Part model, mm, in its own coordinate system. A direction names the side the tool comes from. Round coordinates to 2 decimals unless told otherwise and drop trailing zeros. Order: outer loops, then holes, each group sorted by start corner. A loop starts at its lowest first (then second) coordinate and runs counter-clockwise, first axis right, second up. Notation, with made-up numbers: (14.25, 51.25) - (49.25, 51.25) arc R29 ccw to (49.25, 83.25) - close; hole circle Ø2 at (32.25, -4). An arc over 180 degrees is marked (long way). Return JSON: item names as keys, results as strings. Group by question number.
Item 1: Probe probe 1 along X at (y, z) = (200, -2); probe 2 along Y at (x, z) = (70, -2.2); probe 3 along Y at (x, z) = (-70, -0.55). List the from-to ranges inside material, lowest first.
Item 2: Two-plate mould, pull along Y, no slides. Class faces 4 (the face through (3.21, -127.703, -149.421)), 5 (the face through (200.455, 2.476, -113.421)), 6 (the face through (-3, -200, -3)): released by +Y, released by -Y, zero draft, split by the parting line, or undercut.
Item 3: Saw through at D-D on z = -160.5. List the corners of the cut face in (x, y) (3 decimals), and give its area (3 significant figures).
Item 4: Saw through at B-B on x = -24.5. List the corners of the cut face in (y, z), and give its area (3 significant figures).
Item 5: Tool access for faces 1 (the face through (-1, 180, 0)), 2 (the face through (-3, 200, -3)), 3 (the face through (-200.455, -2.476, -113.421)): list every direction of +Z, -Z, +X, -X, +Y, -Y with a clear straight run to the whole face (end or side of a thin tool).
Item 6: Saw through at A-A on y = 16.5. List the corners of the cut face in (x, z), and give its area (3 significant figures).
Item 7: Saw through at C-C on z = -221.5. List the corners of the cut face in (x, y) (3 decimals), and give its area (3 significant figures).
Item 8: Drop flat-ended pins along their axis: pin 1 (2.5 mm diameter, centred on y = 5, z = -298.5, fed in from -X); pin 2 (1 mm diameter, centred on y = 22.5, z = -248, fed in from +X); pin 3 (0.9 mm diameter, centred on x = 1.5, z = -299, fed in from -Y); pin 4 (9 mm diameter, centred on x = -210, y = -200, fed in from +Z). Give the stop position or say it passes through.
```python
from build123d import *

# Parameters (mm, degrees)
SKETCH1_W                = 460
SKETCH1_H                = 360
BOSS_EXTRUDE1_DEPTH      = 300
CUT_EXTRUDE1_DEPTH       = 578.927331072
CUT_EXTRUDE3_DEPTH       = 302
SHELL1_T                 = -3
SKETCH7_W                = 315.23883128
SKETCH7_H                = 145.74311397
CUT_EXTRUDE4_DEPTH       = 417.544115311
SKETCH8_W                = 460
SKETCH8_H                = 40
BOSS_EXTRUDE2_DEPTH      = 3
BOSS_EXTRUDE3_REACH      = 524.015
SKETCH9_W                = 460
SKETCH9_H                = 3
SKETCH10_W               = 460
SKETCH10_H               = 40
BOSS_EXTRUDE4_DEPTH      = 3
BOSS_EXTRUDE5_REACH      = 552.364
SKETCH11_W               = 460
SKETCH11_H               = 3
F_7_0_7_DIAMETER_HOLE1_D = 7
LPATTERN1_COUNT          = 4
LPATTERN1_PITCH          = 140
MIRROR5_COPY_1_D         = 7
MIRROR5_COPY_2_D         = 7
MIRROR5_COPY_3_D         = 7


with BuildPart() as part:
    # Sketch1 → Boss-Extrude1 (new body)
    with BuildSketch(Plane.XY):
        Rectangle(SKETCH1_W, SKETCH1_H)
    extrude(amount=-BOSS_EXTRUDE1_DEPTH)

    # Sketch3 → Cut-Extrude1 (cut, through all)
    with BuildSketch(Plane(origin=(230, 0, 0), x_dir=(0, 0, -1), z_dir=(1, 0, 0))):
        Polygon((0, 180), (300, 75), (300, 180), align=None)
        Polygon((300, -180), (0, -180), (300, -75), align=None)
    extrude(amount=-CUT_EXTRUDE1_DEPTH, mode=Mode.SUBTRACT)

    # Sketch6 → Cut-Extrude3 (cut, symmetric)
    with BuildSketch(Plane(origin=(0, 0, 0), x_dir=(1, 0, 0), z_dir=(0, 1, 0))):
        Polygon((-230, 0), (-160, 300), (-230, 300), align=None)
        Polygon((230, 300), (230, 0), (160, 300), align=None)
    extrude(amount=CUT_EXTRUDE3_DEPTH, both=True, mode=Mode.SUBTRACT)

    # Shell1
    shell1_openings = [part.faces().sort_by_distance(p)[0] for p in [
        (0, 0, 0),
    ]]
    offset(amount=SHELL1_T, openings=shell1_openings, kind=Kind.INTERSECTION)

    # Sketch7 → Cut-Extrude4 (cut, through all)
    with BuildSketch(Plane.XY.offset(-297)):
        Rectangle(SKETCH7_W, SKETCH7_H)
    extrude(amount=-CUT_EXTRUDE4_DEPTH, mode=Mode.SUBTRACT)

    # Boss-Extrude3: up to this face of the body (flat: up to its plane)
    boss_extrude3_end = Plane(part.part.faces().sort_by_distance((0, -130.641025641, -141.025641026))[0])
    # Sketch9 → Boss-Extrude3 (add, up to the picked face)
    with BuildSketch(Plane(origin=(0, -180, 0), x_dir=(1, 0, 0), z_dir=(0, 1, 0)), mode=Mode.PRIVATE) as boss_extrude3_sk1:
        with Locations((0, 1.5)):
            Rectangle(SKETCH9_W, SKETCH9_H)
    boss_extrude3_tool1 = split(extrude(boss_extrude3_sk1.sketch, amount=BOSS_EXTRUDE3_REACH, mode=Mode.PRIVATE), bisect_by=boss_extrude3_end, keep=Keep.BOTH, mode=Mode.PRIVATE)


with BuildPart() as body_2:
    # Sketch8 → Boss-Extrude2 (new body)
    with BuildSketch(Plane.XY):
        with Locations((0, -200)):
            Rectangle(SKETCH8_W, SKETCH8_H)
    extrude(amount=-BOSS_EXTRUDE2_DEPTH)


with BuildPart() as part_1:
    add(part.part)

    add(body_2.part)  # Boss-Extrude3 merges body 2
    add(boss_extrude3_tool1.solids().sort_by(Axis((0, -180, -1.5), (0, 1, 0)))[0])

    # Boss-Extrude5: up to this face of the body (flat: up to its plane)
    boss_extrude5_end = Plane(part_1.part.faces().sort_by_distance((0, 130.641025641, -141.025641026))[0])
    # Sketch11 → Boss-Extrude5 (add, up to the picked face)
    with BuildSketch(Plane.XZ.offset(-180), mode=Mode.PRIVATE) as boss_extrude5_sk1:
        with Locations((0, -1.5)):
            Rectangle(SKETCH11_W, SKETCH11_H)
    boss_extrude5_tool1 = split(extrude(boss_extrude5_sk1.sketch, amount=BOSS_EXTRUDE5_REACH, mode=Mode.PRIVATE), bisect_by=boss_extrude5_end, keep=Keep.BOTH, mode=Mode.PRIVATE)


with BuildPart() as body_2_2:
    # Sketch10 → Boss-Extrude4 (new body)
    with BuildSketch(Plane.XY):
        with Locations((0, 200)):
            Rectangle(SKETCH10_W, SKETCH10_H)
    extrude(amount=-BOSS_EXTRUDE4_DEPTH)


with BuildPart() as part_2:
    add(part_1.part)

    add(body_2_2.part)  # Boss-Extrude5 merges body 2 2
    add(boss_extrude5_tool1.solids().sort_by(Axis((0, 180, -1.5), (0, -1, 0)))[0])

    # Ø7.0 (7) Diameter Hole1 (through all)
    with Locations(Plane.XY):
        with Locations((-210, 200)):
            f_7_0_7_diameter_hole1 = Hole(F_7_0_7_DIAMETER_HOLE1_D / 2)

    # LPattern1: Ø7.0 (7) Diameter Hole1 ×4
    with Locations(*[(i * LPATTERN1_PITCH, 0, 0) for i in range(1, LPATTERN1_COUNT)]):
        add(f_7_0_7_diameter_hole1, mode=Mode.SUBTRACT)

    # Mirror5: Ø7.0 (7) Diameter Hole1 across plane
    add(f_7_0_7_diameter_hole1.mirror(Plane.ZX), mode=Mode.SUBTRACT)

    # Mirror5 copy 1 (through all)
    with Locations(Plane(origin=(140, 0, 0), x_dir=(1, 0, 0), z_dir=(0, 0, 1))):
        with Locations((-210, -200)):
            Hole(MIRROR5_COPY_1_D / 2)

    # Mirror5 copy 2 (through all)
    with Locations(Plane(origin=(280, 0, 0), x_dir=(1, 0, 0), z_dir=(0, 0, 1))):
        with Locations((-210, -200)):
            Hole(MIRROR5_COPY_2_D / 2)

    # Mirror5 copy 3 (through all)
    with Locations(Plane(origin=(420, 0, 0), x_dir=(1, 0, 0), z_dir=(0, 0, 1))):
        with Locations((-210, -200)):
            Hole(MIRROR5_COPY_3_D / 2)


solid = part_2.part
```
Filled in:
{
 "1": {"probe 1": "x = -230 to -213.5, -206.5 to -73.5, -66.5 to 66.5, 73.5 to 206.5, 213.5 to 230", "probe 2": "y = -220 to -203.5, -196.5 to -176.05, 176.05 to 196.5, 203.5 to 220", "probe 3": "y = -220 to -203.5, -196.5 to -176.63, 176.63 to 196.5, 203.5 to 220"},
 "2": {"face 4": "released by -Y", "face 5": "undercut", "face 6": "zero draft"},
 "3": {"outline": "(-192.55, -123.825) - (192.55, -123.825) - (192.55, 123.825) - (-192.55, 123.825) - close; hole (-189.469, -120.647) - (189.469, -120.647) - (189.469, 120.647) - (-189.469, 120.647) - close", "area": "3,930 mm^2"},
 "4": {"outline": "(-220, -3) - (-178.95, -3) - (-75, -300) - (-72.87, -300) - (-72.87, -297) - (-176.82, 0) - (-220, 0) - close; (72.87, -300) - (75, -300) - (178.95, -3) - (220, -3) - (220, 0) - (176.82, 0) - (72.87, -297) - close", "area": "2,150 mm^2"},
 "5": {"face 1": "+Z, +X, -X, +Y, -Y", "face 2": "-Z, +X, -X, +Y", "face 3": "+Z"},
 "6": {"outline": "(-230, 0) - (-160, -300) - (-157.62, -300) - (-157.62, -297) - (-226.92, 0) - close; (157.62, -300) - (160, -300) - (230, 0) - (226.92, 0) - (157.62, -297) - close", "area": "1,850 mm^2"},
 "7": {"outline": "(-178.317, -102.475) - (178.317, -102.475) - (178.317, 102.475) - (-178.317, 102.475) - close; hole (-175.236, -99.297) - (175.236, -99.297) - (175.236, 99.297) - (-175.236, 99.297) - close", "area": "3,490 mm^2"},
 "8": {"pin 1": "stops at x = -160.64", "pin 2": "stops at x = 172.25", "pin 3": "stops at y = -75.51", "pin 4": "stops at z = 0"}
}
